from build123d import *

# Parameters (mm, degrees)
SKETCH2_R          = 10.25
CUT_EXTRUDE1_DEPTH = 56.713553109
SKETCH4_R          = 12.188770661
CUT_EXTRUDE2_DEPTH = 20


with BuildPart() as part:
    # Sketch1 → Revolve1 (revolve)
    with BuildSketch(Plane.XY):
        Polygon((-48, 0), (-48, 15.5), (-47, 16.5), (-23, 16.5), (-23, 20), (-13, 20), (-13, 17.5), (0, 17.5), (0, 0), align=None)
    revolve(axis=Axis((0, 0, 0), (-1, 0, 0)))

    # Sketch2 → Cut-Extrude1 (cut, through all)
    with BuildSketch(Plane(origin=(0, 0, 0), x_dir=(0, 0, -1), z_dir=(1, 0, 0))):
        with Locations(Location((0, 0, 0), (0, 0, 90))):
            Circle(SKETCH2_R)
    extrude(amount=-CUT_EXTRUDE1_DEPTH, mode=Mode.SUBTRACT)

    # Sketch4 → Cut-Extrude2 (cut)
    with BuildSketch(Plane(origin=(0, 0, 0), x_dir=(0, 0, -1), z_dir=(1, 0, 0))):
        with Locations(Location((0, 0, 0), (0, 0, 90))):
            Circle(SKETCH4_R)
    extrude(amount=-CUT_EXTRUDE2_DEPTH, mode=Mode.SUBTRACT)


solid = part.part
For this review, take the finished solid that the model builds, in its own axes (mm). A direction names the side the tool comes from. Give positions to 0.01 mm unless a question says otherwise; leave off trailing zeros. Loops run counter-clockwise (first coordinate to the right, second up) from the corner with the lowest first, then second, coordinate; pieces in that order, holes last. Notation, with made-up numbers: (48.25, 50.25) - (77.25, 50.25) arc R23 cw to (77.25, 61.25) - close; hole circle Ø4 at (45.5, 2.5). An arc over 180 degrees is marked (long way). Write each question's results on one line, items separated by ' | '.
(1) For pin 1 Ø8 at (x, z) = (-31.5, 1.5) entering from -Y; pin 2 Ø1.5 at (x, y) = (-16.5, -9) entering from +Z; pin 3 Ø2 at (x, z) = (-16, -9.5) entering from -Y, all flat-tipped, find the tip position at first contact; note any pin that passes through.
Conclusion:
pin 1: y = -16.5 | pin 2: z = 18.22 | pin 3: y = -18.1
(2) Take a section at A-A (y = 0). Give the boundary of the cut face in (x, z).
Conclusion:
outline: (-48, -15.5) - (-47, -16.5) - (-23, -16.5) - (-23, -20) - (-13, -20) - (-13, -17.5) - (0, -17.5) - (0, -12.19) - (-20, -12.19) - (-20, -10.25) - (-48, -10.25) - close; (-48, 10.25) - (-20, 10.25) - (-20, 12.19) - (0, 12.19) - (0, 17.5) - (-13, 17.5) - (-13, 20) - (-23, 20) - (-23, 16.5) - (-47, 16.5) - (-48, 15.5) - close
(3) Draft analysis for pull direction Z (two halves, no side actions). For faces 4 (the cylindrical face through (-6.409, -13.887, 10.648)), 5 (the flat face through (0, -12, 4)), 6 (the cylindrical face through (-9.86, 11.626, 3.661)), state which applies: +Z half, -Z half, draft (parallel to the pull), parting line (faces both ways), or undercut.
Conclusion:
face 4: parting line | face 5: draft | face 6: undercut
(4) Take a section at C-C (x = -9.5). Give the boundary of the cut face in (y, z), then the cut area to 3 significant figures.
Conclusion:
outline: circle Ø35 at (0, 0); hole circle Ø24.38 at (0, 0) | area: 495 mm^2
(5) For line 1 along Z through (x, y) = (-30.25, 0); line 2 along Z through (x, y) = (-15, 0); line 3 along Y through (x, z) = (-32.5, -0.5), list the stretches that pass through material, from the lowest coordinate up.
Conclusion:
line 1: -16.5 to -10.25, 10.25 to 16.5 | line 2: -20 to -12.19, 12.19 to 20 | line 3: -16.49 to -10.24, 10.24 to 16.49
(6) For faces 1 (the flat face through (-23, -2.9, -16.4)), 2 (the cylindrical face through (-33.804, -2.222, -10.006)), 3 (the flat face through (-13, 0, 18)), list the 3-axis set-ups (+Z, -Z, +X, -X, +Y, -Y) from which the entire face can be reached by the end or side of a thin tool; tool diameter is ignored.
Conclusion:
face 1: -X | face 2: +X, -X | face 3: +X
